Geometry: final body of the model. Coordinates: model frame, mm. A direction names the side the tool comes from. Round coordinates to 2 decimals unless told otherwise and drop trailing zeros. Write each loop counter-clockwise with the first axis right and the second up, starting at its lowest first coordinate (ties: lowest second). Pieces come first, ordered by that corner, then holes.
from build123d import *

# Parameters (mm, degrees)
EXTRUDE_1_DEPTH     = 6
SKETCH_2_R          = 1.5
EXTRUDE_2_DEPTH     = 6
SKETCH_3_R          = 1.5
CUT_EXTRUDE_1_DEPTH = 3


with BuildPart() as part:
    # 草图1 → 凸台-拉伸1 (new body)
    with BuildSketch(Plane.XY):
        Polygon((3.464101615, 0), (1.732050808, 3), (-1.732050808, 3), (-3.464101615, 0), (-1.732050808, -3), (1.732050808, -3), align=None)
    extrude(amount=EXTRUDE_1_DEPTH)

    # 草图2 → 凸台-拉伸2 (add)
    with BuildSketch(Plane.XY.offset(6)):
        Circle(SKETCH_2_R)
    extrude(amount=EXTRUDE_2_DEPTH)

    # 草图3 → 切除-拉伸1 (cut)
    with BuildSketch(Plane(origin=(0, 0, 0), x_dir=(-1, 0, 0), z_dir=(0, 0, -1))):
        with Locations(Location((0, 0, 0), (0, 0, 180))):
            Circle(SKETCH_3_R)
    extrude(amount=-CUT_EXTRUDE_1_DEPTH, mode=Mode.SUBTRACT)


solid = part.part
1) Draft query along X for faces 4 (the flat face through (0, 0, 3)), 5 (the flat face through (2.6, 1.5, 3)), 6 (the flat face through (1.5, 0.7, 0)). Return one class per face: pulls with the +X half, pulls with the -X half, needs draft (parallel to the pull), parting line crosses it, or undercut.
2) First-contact query: P1, Ø3, axis at y = 1.5, z = 10, coming from the -X side. Flat tip, straight axial feed; report the tip coordinate or a pass-through.
3) Section A-A on x = 0. Output: boundary loops of the cut face in (y, z).
4) Section D-D on x = 2.75. Output: boundary loops of the cut face in (y, z), plus the area to 3 significant figures.
5) Line query: probe 1 along Y at (x, z) = (0, 1.9); probe 2 along Z at (x, y) = (-0.25, -1); probe 3 along Z at (x, y) = (-2.75, -0.5). Output: solid intervals per line, ascending.
6) Section B-B on y = 0.5. Output: boundary loops of the cut face in (x, z).
7) Reachability of faces 1 (the cylindrical face through (-1.5, 0.07, 8.96)), 2 (the cylindrical face through (1.43, -0.45, 1.48)), 3 (the flat face through (-2.6, 1.5, 3)) from +Z, -Z, +X, -X, +Y, -Y: full face, straight path, thin tool, end or side. Return the list, or none.
8) Section C-C on z = 10. Output: boundary loops of the cut face in (x, y), plus the area to 3 significant figures.
Filled in:
1. face 4: undercut
1. face 5: pulls with the +X half
1. face 6: needs draft
2. P1: stops at x = -1.5
3. outline: (-3, 0) - (-1.5, 0) - (-1.5, 3) - (1.5, 3) - (1.5, 0) - (3, 0) - (3, 6) - (1.5, 6) - (1.5, 12) - (-1.5, 12) - (-1.5, 6) - (-3, 6) - close
4. outline: (-1.24, 0) - (1.24, 0) - (1.24, 6) - (-1.24, 6) - close
4. area: 14.8 mm2
5. probe 1: y = -3 to -1.5, 1.5 to 3
5. probe 2: z = 3 to 12
5. probe 3: z = 0 to 6
6. outline: (-3.18, 0) - (-1.41, 0) - (-1.41, 3) - (1.41, 3) - (1.41, 0) - (3.18, 0) - (3.18, 6) - (1.41, 6) - (1.41, 12) - (-1.41, 12) - (-1.41, 6) - (-3.18, 6) - close
7. face 1: +Z
7. face 2: -Z
7. face 3: +Z, -Z, -X, +Y
8. outline: circle Ø3 at (0, 0)
8. area: 7.07 mm2
